from build123d import *

# Parameters (mm, degrees)
FLANGE_BOLT_HOLES_4X_10_REACH = 93.788
FLANGE_BOLT_HOLES_SKETCH_R    = 5
BEARING_START                 = 60
BEARING_BLOCK_DEPTH           = 60
SPLIT_CAP_LUGS_SKETCH_R       = 8
SPLIT_CAP_LUGS_DEPTH          = 30
JOURNAL_SEAT_SPLIT_CUT_REACH  = 141.718


with BuildPart() as part:
    # Flanged Hub Profile → Flanged Hub (revolve)
    with BuildSketch(Plane.XY):
        Polygon((0, 60), (-35, 60), (-35, 30), (-65, 30), (-65, 12.5), (-15, 12.5), (-15, 55), (0, 55), align=None)
    revolve(axis=Axis((0, 0, 0), (-1, 0, 0)))

    # Flange Bolt Holes Sketch → Flange Bolt Holes 4xØ10 (cut, up to next)
    with BuildSketch(Plane.ZY.offset(35), mode=Mode.PRIVATE) as flange_bolt_holes_4x_10_sk1:
        with Locations(Location((42, 0, 0), (0, 0, 270))):
            Circle(FLANGE_BOLT_HOLES_SKETCH_R)
    flange_bolt_holes_4x_10_tool1 = extrude(flange_bolt_holes_4x_10_sk1.sketch, amount=-FLANGE_BOLT_HOLES_4X_10_REACH, mode=Mode.PRIVATE) & part.part
    # Flange Bolt Holes Sketch → Flange Bolt Holes 4xØ10 (cut, up to next)
    with BuildSketch(Plane.ZY.offset(35), mode=Mode.PRIVATE) as flange_bolt_holes_4x_10_sk2:
        with Locations(Location((0, -42, 0), (0, 0, 270))):
            Circle(FLANGE_BOLT_HOLES_SKETCH_R)
    flange_bolt_holes_4x_10_tool2 = extrude(flange_bolt_holes_4x_10_sk2.sketch, amount=-FLANGE_BOLT_HOLES_4X_10_REACH, mode=Mode.PRIVATE) & part.part
    # Flange Bolt Holes Sketch → Flange Bolt Holes 4xØ10 (cut, up to next)
    with BuildSketch(Plane.ZY.offset(35), mode=Mode.PRIVATE) as flange_bolt_holes_4x_10_sk3:
        with Locations(Location((-42, 0, 0), (0, 0, 270))):
            Circle(FLANGE_BOLT_HOLES_SKETCH_R)
    flange_bolt_holes_4x_10_tool3 = extrude(flange_bolt_holes_4x_10_sk3.sketch, amount=-FLANGE_BOLT_HOLES_4X_10_REACH, mode=Mode.PRIVATE) & part.part
    # Flange Bolt Holes Sketch → Flange Bolt Holes 4xØ10 (cut, up to next)
    with BuildSketch(Plane.ZY.offset(35), mode=Mode.PRIVATE) as flange_bolt_holes_4x_10_sk4:
        with Locations(Location((0, 42, 0), (0, 0, 270))):
            Circle(FLANGE_BOLT_HOLES_SKETCH_R)
    flange_bolt_holes_4x_10_tool4 = extrude(flange_bolt_holes_4x_10_sk4.sketch, amount=-FLANGE_BOLT_HOLES_4X_10_REACH, mode=Mode.PRIVATE) & part.part
    add(flange_bolt_holes_4x_10_tool1.solids().sort_by_distance((-35, 0, 42))[0], mode=Mode.SUBTRACT)
    add(flange_bolt_holes_4x_10_tool2.solids().sort_by_distance((-35, -42, 0))[0], mode=Mode.SUBTRACT)
    add(flange_bolt_holes_4x_10_tool3.solids().sort_by_distance((-35, 0, -42))[0], mode=Mode.SUBTRACT)
    add(flange_bolt_holes_4x_10_tool4.solids().sort_by_distance((-35, 42, 0))[0], mode=Mode.SUBTRACT)

    # Bearing Block Sketch → Bearing Block (add)
    with BuildSketch(Plane.ZY.offset(65).offset(BEARING_START)):
        with BuildLine():
            Line((-30, 0), (-20, 0))
            ThreePointArc((-20, 0), (0, -20), (20, 0))
            Line((20, 0), (30, 0))
            ThreePointArc((30, 0), (0, -30), (-30, 0))
        make_face()
    extrude(amount=-BEARING_BLOCK_DEPTH)

    # Split Cap Lugs Sketch → Split Cap Lugs (add)
    with BuildSketch(Plane(origin=(0, 0, 0), x_dir=(1, 0, 0), z_dir=(0, 1, 0))):
        with BuildLine():
            Line((-111, -44), (-111, 44))
            ThreePointArc((-111, 44), (-95, 60), (-79, 44))
            Line((-79, 44), (-79, -44))
            ThreePointArc((-79, -44), (-95, -60), (-111, -44))
        make_face()
        with Locations(Location((-95, 44, 0), (0, 0, 180))):
            Circle(SPLIT_CAP_LUGS_SKETCH_R, mode=Mode.SUBTRACT)
        with Locations(Location((-95, -44, 0), (0, 0, 180))):
            Circle(SPLIT_CAP_LUGS_SKETCH_R, mode=Mode.SUBTRACT)
    extrude(amount=-SPLIT_CAP_LUGS_DEPTH)

    # Journal Seat Split Sketch → Journal Seat Split Cut (cut, up to next)
    with BuildSketch(Plane.ZY.offset(111), mode=Mode.PRIVATE) as journal_seat_split_cut_sk1:
        with BuildLine():
            Line((20, 0), (-20, 0))
            ThreePointArc((-20, 0), (0, -20), (20, 0))
        make_face()
    journal_seat_split_cut_tool1 = extrude(journal_seat_split_cut_sk1.sketch, amount=-JOURNAL_SEAT_SPLIT_CUT_REACH, mode=Mode.PRIVATE) & part.part
    add(journal_seat_split_cut_tool1.solids().sort_by_distance((-111, -8.488264, 0))[0], mode=Mode.SUBTRACT)


solid = part.part
Verification items for the finished model (mm, model axes). A direction names the side the tool comes from. Coordinates: 2 decimals unless noted, no trailing zeros. Order: outer loops, then holes, each group sorted by start corner. A loop starts at its lowest first (then second) coordinate and runs counter-clockwise, first axis right, second up.
1. Sectioned sample at C-C, the plane z = 39.5. Record the cut outline in (x, y), and give its area (3 significant figures).
Results found:
outline: (-111, -30) - (-101.61, -30) - (-101.61, 0) - (-111, 0) - close; (-88.39, -30) - (-79, -30) - (-79, 0) - (-88.39, 0) - close; (-35, -45.16) - (0, -45.16) - (0, -38.27) - (-15, -38.27) - (-15, -4.33) - (-35, -4.33) - close; (-35, 4.33) - (-15, 4.33) - (-15, 38.27) - (0, 38.27) - (0, 45.16) - (-35, 45.16) - close
area: 2,400 mm2
2. Sectioned sample at A-A, the plane x = -95. Record the cut outline in (y, z), and give its area (3 significant figures).
Results found:
outline: (-30, -60) - (0, -60) - (0, -52) - (-30, -52) - close; (-30, -36) - (0, -36) - (0, -20) arc R20 cw to (0, 20) - (0, 36) - (-30, 36) - close; (-30, 52) - (0, 52) - (0, 60) - (-30, 60) - close
area: 2,010 mm2
3. Sectioned sample at B-B, the plane y = 42. Record the cut outline in (x, z).
Results found:
outline: (-35, -42.85) - (0, -42.85) - (0, -35.51) - (-15, -35.51) - (-15, -5) - (-35, -5) - close; (-35, 5) - (-15, 5) - (-15, 35.51) - (0, 35.51) - (0, 42.85) - (-35, 42.85) - close
4. Go/stop test with flat-tipped pins: pin 1 Ø24 at (y, z) = (-13.5, -28) entering from +X; pin 2 Ø11.5 at (y, z) = (42, 0) entering from -X; pin 3 Ø24 at (y, z) = (-15, 29) entering from -X; pin 4 Ø12 at (x, z) = (-105.5, 25) entering from -Y. Record where each tip stops, or that it passes through.
Results found:
pin 1: stops at x = -15
pin 2: stops at x = -35
pin 3: stops at x = -125
pin 4: stops at y = -30
5. Scan lines: line 1 (Z direction, x = -29, y = 0); line 2 (Z direction, x = -95, y = -10.5); line 3 (X direction, y = -23, z = -23). Record each from-to range of solid material in increasing order.
Results found:
line 1: z = -60 to -47, -37 to -12.5, 12.5 to 37, 47 to 60
line 2: z = -60 to -52, -36 to -17.02, 17.02 to 36, 52 to 60
line 3: x = -111 to -79, -35 to -15
6. Release check for a two-part mould opening along X. For faces 5 (the face through (-95, 0, 35)), 6 (the face through (-79, -18, 31)), 7 (the face through (-35, 12, -28)), 8 (the face through (-15, 1, -13)) record: +X half, -X half, draft (parallel to the pull), parting line (faces both ways), or undercut.
Results found:
face 5: draft
face 6: undercut
face 7: undercut
face 8: +X half
7. Set-up check for faces 1 (the face through (-25.14, 0.651, -37.043)), 2 (the face through (-111, -18, 32)), 3 (the face through (-94.6, 0, -35.8)), 4 (the face through (-65, 16, 0)): record each of +Z, -Z, +X, -X, +Y, -Y from which the full face is reachable in a straight line by a thin tool's end or side.
Results found:
face 1: +X
face 2: +Z, -X, -Y
face 3: +Z, -Z, -X, +Y
face 4: -X, +Y
8. Sectioned sample at D-D, the plane x = -50. Record the cut outline in (y, z).
Results found:
outline: circle Ø60 at (0, 0); hole circle Ø25 at (0, 0)
